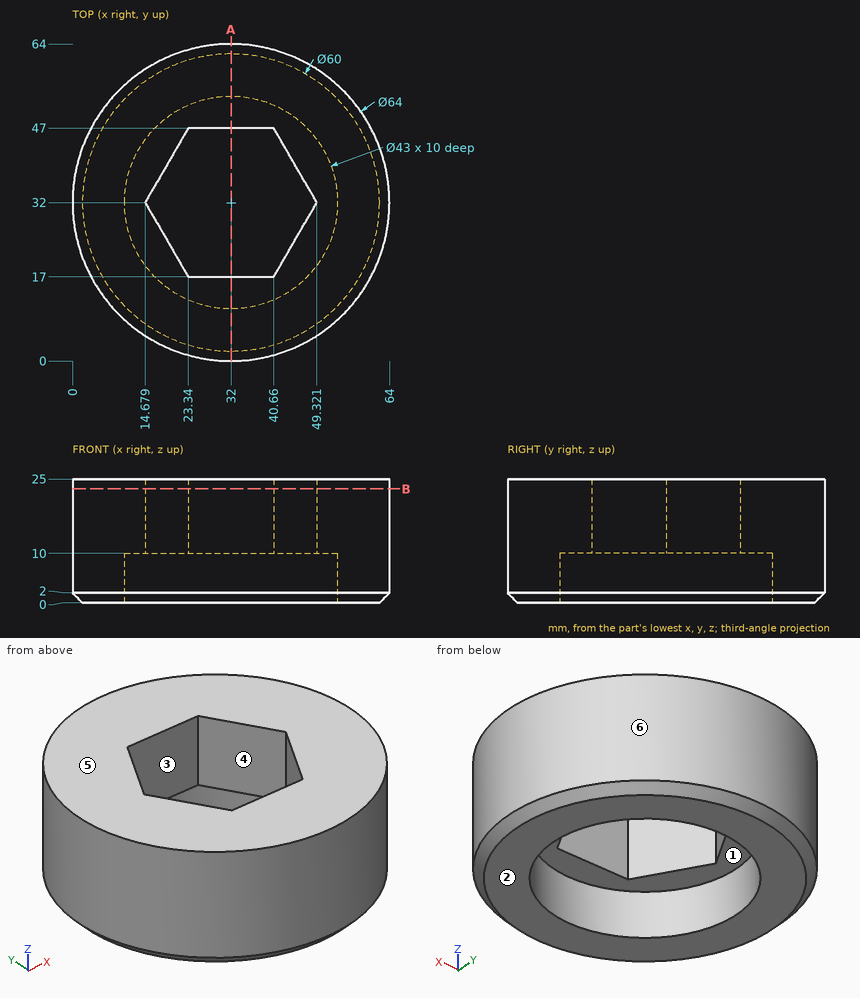
Geometry check sheet. Reference: drawing and pictorial views, mm from the part's lowest x, y, z. A direction names the side the tool comes from. Round coordinates to 2 decimals unless told otherwise and drop trailing zeros. Write each loop counter-clockwise with the first axis right and the second up, starting at its lowest first coordinate (ties: lowest second). Pieces come first, ordered by that corner, then holes.
1. Draft check along X on the marked faces 4, 5 and 6. Enter one of: +X half, -X half, draft (parallel to the pull), parting line (faces both ways), or undercut.
2. Section check A-A on x = 32. Enter the section's corners in (y, z).
3. Access from +Z, -Z, +X, -X, +Y, -Y to the whole of each face (thin tool, end or side, straight path). Record for the marked faces 1, 2 and 3.
4. Section check B-B on z = 23. Enter the section's corners in (x, y), plus the area to 3 significant figures.
5. Scan lines: L1, parallel to Y at x = 32, z = 8.25; L2, parallel to Z at x = 27, y = 48; L3, parallel to Y at x = 27, z = 3. Record each from-to range of solid material in increasing order.
6. Gauge pin test, flat ends, axial feed: P1, Ø7.5, axis at x = 33, z = 16, coming from the -Y side; P2, Ø12, axis at x = 36, z = 20, coming from the +Y side; P3, Ø1, axis at x = 25.5, z = 15.5, coming from the -Y side. Record the tip position at first contact, or that the pin passes through.
Answer:
1. face 4: undercut
1. face 5: draft
1. face 6: parting line
2. outline: (0, 2) - (2, 0) - (10.5, 0) - (10.5, 10) - (17, 10) - (17, 25) - (0, 25) - close; (47, 10) - (53.5, 10) - (53.5, 0) - (62, 0) - (64, 2) - (64, 25) - (47, 25) - close
3. face 1: -Z
3. face 2: -Z, +X, -X, +Y, -Y
3. face 3: +Z, -Z
4. outline: circle Ø64 at (32, 32); hole (14.68, 32) - (23.34, 17) - (40.66, 17) - (49.32, 32) - (40.66, 47) - (23.34, 47) - close
4. area: 2,440 mm2
5. L1: y = 0 to 10.5, 53.5 to 64
5. L2: z = 10 to 25
5. L3: y = 0.39 to 11.09, 52.91 to 63.61
6. P1: stops at y = 0
6. P2: stops at y = 64
6. P3: stops at y = 0.57
